```python
from build123d import *

# Parameters (mm, degrees)
SKETCH_1_W          = 250
SKETCH_1_H          = 40
EXTRUDE_1_DEPTH     = 5
SKETCH_2_W          = 60
SKETCH_2_H          = 40
CUT_EXTRUDE_1_DEPTH = 2


with BuildPart() as part:
    # 草图1 → 凸台-拉伸1 (new, symmetric)
    with BuildSketch(Plane.XY):
        Rectangle(SKETCH_1_W, SKETCH_1_H)
    extrude(amount=EXTRUDE_1_DEPTH, both=True)

    # 草图2 → 切除-拉伸1 (cut)
    with BuildSketch(Plane(origin=(0, 0, -5), x_dir=(-1, 0, 0), z_dir=(0, 0, -1))):
        with Locations((95, 0)):
            Rectangle(SKETCH_2_W, SKETCH_2_H)
    extrude(amount=-CUT_EXTRUDE_1_DEPTH, mode=Mode.SUBTRACT)


solid = part.part
```
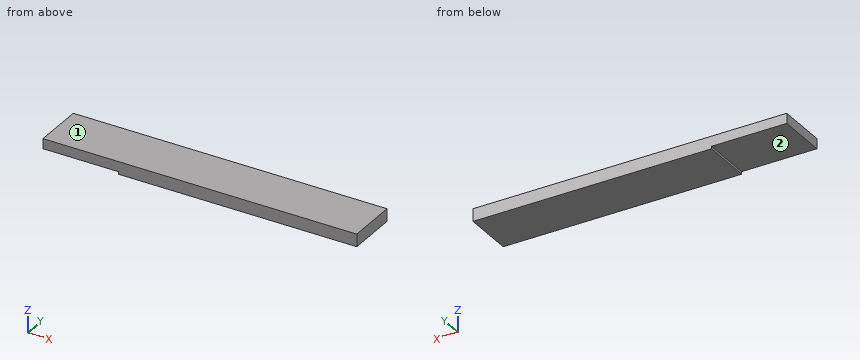
For this review, take the finished solid that the model builds, in its own axes (mm). Face numbers are marked on the shaded views. A direction names the side the tool comes from. Round coordinates to 2 decimals unless told otherwise and drop trailing zeros. Write each loop counter-clockwise with the first axis right and the second up, starting at its lowest first coordinate (ties: lowest second). Pieces come first, ordered by that corner, then holes. Notation, with made-up numbers: (-33.5, -32) -> (-22.5, -32) arc R25 cw to (-22.5, -13) -> close; hole circle Ø11 at (71, 41.5). An arc over 180 degrees is marked (long way). Use one line per item in the form item = value.
1) Take a section at A-A, the plane y = 4.5. Write out the cut boundary in (x, z).
Found:
outline = (-125, -3) -> (-65, -3) -> (-65, -5) -> (125, -5) -> (125, 5) -> (-125, 5) -> close
2) To check wall thickness, follow L1, parallel to X at y = -4.5, z = -3.5; L2, parallel to Z at x = -101.5, y = 3.5. State the ranges of each line that lie inside material, in increasing order. Write a range as from..to.
Found:
L1 = -65..125
L2 = -3..5
3) Tool access review of the marked faces 1 and 2: name each direction out of +Z, -Z, +X, -X, +Y, -Y from which nothing blocks a thin tool from reaching the whole face with its end or side.
Found:
face_1 = +Z, +X, -X, +Y, -Y
face_2 = -Z, -X, +Y, -Y
4) Take a section at B-B, the plane x = -105.5. Write out the cut boundary in (y, z).
Found:
outline = (-20, -3) -> (20, -3) -> (20, 5) -> (-20, 5) -> close
